```python
from build123d import *

# Parameters (mm, degrees)
SKETCH1_R          = 6.9175
BOSS_EXTRUDE_DEPTH = 15.9
SKETCH2_OUTSIDE_W  = 120.762
SKETCH2_OUTSIDE_H  = 117.252
SKETCH2_OUTSIDE_R  = 11.34493279
CUT_EXTRUDE1_DEPTH = 24.518662802
CUT_EXTRUDE1_DRAFT = -60
SKETCH3_OUTSIDE_W  = 120.762
SKETCH3_OUTSIDE_H  = 117.252
SKETCH3_OUTSIDE_R  = 11.34493279
CUT_EXTRUDE2_DEPTH = 24.518662802
CUT_EXTRUDE2_DRAFT = -60
CHAMFER1_SIZE      = 0.3975


with BuildPart() as part:
    # Sketch1 → Boss-Extrude (new body)
    with BuildSketch(Plane.XY):
        Polygon((6.55, 11.34493279), (-6.55, 11.34493279), (-13.1, 0), (-6.55, -11.34493279), (6.55, -11.34493279), (13.1, 0), align=None)
        Circle(SKETCH1_R, mode=Mode.SUBTRACT)
    extrude(amount=BOSS_EXTRUDE_DEPTH)


with BuildPart() as cut_extrude1_tool:
    # Sketch2 outside → Cut-Extrude1 (with draft: the straight prism first)
    with BuildSketch(Plane(origin=(0, 0, 0), x_dir=(-1, 0, 0), z_dir=(0, 0, -1))):
        Rectangle(SKETCH2_OUTSIDE_W, SKETCH2_OUTSIDE_H)
        Circle(SKETCH2_OUTSIDE_R, mode=Mode.SUBTRACT)
    extrude(amount=-CUT_EXTRUDE1_DEPTH)
    # Cut-Extrude1: the draft: its side faces are tilted about the plane it starts from
    cut_extrude1_sides = [cut_extrude1_tool.faces().sort_by_distance(p)[0] for p in [
        (0, -58.626, 12.259331401),
        (-60.381, 0, 12.259331401),
        (0, 58.626, 12.259331401),
        (60.381, 0, 12.259331401),
        (11.34493279, 0, 12.259331401),
    ]]
    draft(cut_extrude1_sides, Plane(origin=(0, 0, 0), x_dir=(-1, 0, 0), z_dir=(0, 0, -1)), CUT_EXTRUDE1_DRAFT)


with BuildPart() as part_1:
    add(part.part)

    # Cut-Extrude1: cut by cut_extrude1_tool
    add(cut_extrude1_tool.part, mode=Mode.SUBTRACT)


with BuildPart() as cut_extrude2_tool:
    # Sketch3 outside → Cut-Extrude2 (with draft: the straight prism first)
    with BuildSketch(Plane.XY.offset(15.9)):
        Rectangle(SKETCH3_OUTSIDE_W, SKETCH3_OUTSIDE_H)
        Circle(SKETCH3_OUTSIDE_R, mode=Mode.SUBTRACT)
    extrude(amount=-CUT_EXTRUDE2_DEPTH)
    # Cut-Extrude2: the draft: its side faces are tilted about the plane it starts from
    cut_extrude2_sides = [cut_extrude2_tool.faces().sort_by_distance(p)[0] for p in [
        (0, -58.626, 3.640668599),
        (60.381, 0, 3.640668599),
        (0, 58.626, 3.640668599),
        (-60.381, 0, 3.640668599),
        (-11.34493279, 0, 3.640668599),
    ]]
    draft(cut_extrude2_sides, Plane.XY.offset(15.9), CUT_EXTRUDE2_DRAFT)


with BuildPart() as part_2:
    add(part_1.part)

    # Cut-Extrude2: cut by cut_extrude2_tool
    add(cut_extrude2_tool.part, mode=Mode.SUBTRACT)

    # Chamfer1
    chamfer1_edges = [part_2.edges().sort_by_distance(p)[0] for p in [
        (-6.9175, 0, 0),
        (-6.9175, 0, 15.9),
    ]]
    chamfer(chamfer1_edges, length=CHAMFER1_SIZE)


solid = part_2.part
```
Check sheet for the modelled part. Datum: model origin and axes. Units: mm. Round coordinates to 2 decimals unless told otherwise and drop trailing zeros. Put each result on its own line as item: value.
(1) Material ranges on line 1 (X direction, y = -3.5, z = 4.25); line 2 (Y direction, x = 1.5, z = 13.25); line 3 (X direction, y = -4.25, z = 13), recorded low to high.
Values found:
line 1: x = -11.08 to -5.97, 5.97 to 11.08
line 2: y = -11.34 to -6.75, 6.75 to 11.34
line 3: x = -10.65 to -5.46, 5.46 to 10.65
(2) Go/stop test with flat-tipped pins: pin 1 Ø4 at (y, z) = (-1, 8) entering from +X; pin 2 Ø5 at (y, z) = (-4.5, 4) entering from +X. Record where each tip stops, or that it passes through.
Values found:
pin 1: stops at x = 13.1
pin 2: stops at x = 11.95
(3) Mould release check, pull along Y, two halves, no side actions. Record for faces 1 (the face through (5.86, 10.2, 0.24)), 2 (the face through (-6.91, 0.3, 7.84)), 3 (the face through (-11.76, -0.03, 0.24)): released by +Y, released by -Y, zero draft, split by the parting line, or undercut.
Values found:
face 1: released by +Y
face 2: undercut
face 3: split by the parting line
